```python
from build123d import *

# Parameters (mm, degrees)
EXTRUDE_1_DEPTH    = 100
SKETCH_2_W         = 6
SKETCH_2_H         = 1
EXTRUDE_2_DEPTH    = 100
HOLE_WIZARD_M3_1_D = 3.4


with BuildPart() as part:
    # 草图1 → 拉伸-薄壁1 (new body)
    with BuildSketch(Plane.XY):
        Polygon((2.35, 5), (0, 5), (0, 0), (8, 0), (8, 5), (5.65, 5), (5.65, 4), (7, 4), (7, 1), (1, 1), (1, 4), (2.35, 4), align=None)
    extrude(amount=EXTRUDE_1_DEPTH)

    # 草图2 → 拉伸-薄壁2 (add)
    with BuildSketch(Plane.XY.offset(100)):
        with Locations((-3, 0.5)):
            Rectangle(SKETCH_2_W, SKETCH_2_H)
    extrude(amount=-EXTRUDE_2_DEPTH)

    # 镜向1: part across plane


with BuildPart() as part_1:
    add(part.part)
    add(part.part.mirror(Plane(origin=(-6, 0, -6.08276253), x_dir=(0, 0, 1), z_dir=(1, 0, 0))))

    # M3 间隙孔1 (through all)
    with Locations(Plane(origin=(0, 1, 0), x_dir=(1, 0, 0), z_dir=(0, 1, 0))):
        with Locations((-6, -90), (-6, -10)):
            Hole(HOLE_WIZARD_M3_1_D / 2)


solid = part_1.part
```
Geometry check sheet. Reference: the model listing, model coordinates, mm. A direction names the side the tool comes from. Round coordinates to 2 decimals unless told otherwise and drop trailing zeros. Loops run counter-clockwise (first coordinate to the right, second up) from the corner with the lowest first, then second, coordinate; pieces in that order, holes last. Notation, with made-up numbers: M 85,-29 L 107,-29 A16 ccw 107,-22 Z; hole C 37.5,61.5 d9. An arc over 180 degrees is marked long. Return JSON: item names as keys, results as strings. Group by question number.
(1) Section check D-D, the plane x = 3.5. Enter the section's corners in (y, z), and give its area (3 significant figures).
(2) Section check C-C, the plane z = 79. Enter the section's corners in (x, y), and give its area (3 significant figures).
(3) Scan lines: line 1 along X through (y, z) = (3.65, 59); line 2 along Z through (x, y) = (-6, 0.75); line 3 along X through (y, z) = (4.25, 11.5). Record each from-to range of solid material in increasing order. Write a range as [from, to].
(4) Set-up check for faces 1 (the face through (0, 3, 49)), 2 (the face through (-19, 3, 49)), 3 (the face through (-5.8, 0.3, 0)): record each of +Z, -Z, +X, -X, +Y, -Y from which the full face is reachable in a straight line by a thin tool's end or side.
(5) Mould release check, pull along Y, two halves, no side actions. Record for faces 4 (the face through (-16, 1, 49)), 5 (the face through (1, 5, 49)), 6 (the face through (-5.63, 0.49, 91.66)): pulls with the +Y half, pulls with the -Y half, needs draft (parallel to the pull), parting line crosses it, or undercut.
(6) Section check A-A, the plane x = -6. Enter the section's corners in (y, z).
(7) Go/stop test with a flat-tipped pin: pin 1 (1.8 mm diameter, centred on x = -15.5, z = 55.5, fed in from +Y). Record where the tip stops, or that it passes through.
(8) Section check B-B, the plane z = 10. Enter the section's corners in (x, y), and give its area (3 significant figures).
Data:
{
 "1": {"outline": "M 0,0 L 1,0 L 1,100 L 0,100 Z", "area": "100 mm²"},
 "2": {"outline": "M -20,0 L 8,0 L 8,5 L 5.65,5 L 5.65,4 L 7,4 L 7,1 L 1,1 L 1,4 L 2.35,4 L 2.35,5 L 0,5 L 0,1 L -12,1 L -12,5 L -14.35,5 L -14.35,4 L -13,4 L -13,1 L -19,1 L -19,4 L -17.65,4 L -17.65,5 L -20,5 Z", "area": "49.4 mm²"},
 "3": {"line 1": "[-20, -19], [-13, -12], [0, 1], [7, 8]", "line 2": "[0, 8.3], [11.7, 88.3], [91.7, 100]", "line 3": "[-20, -17.65], [-14.35, -12], [0, 2.35], [5.65, 8]"},
 "4": {"face 1": "+Z, -Z, +Y", "face 2": "+Z, -Z", "face 3": "-Z, +X, -X, +Y, -Y"},
 "5": {"face 4": "undercut", "face 5": "pulls with the +Y half", "face 6": "needs draft"},
 "6": {"outline": "M 0,0 L 1,0 L 1,8.3 L 0,8.3 Z; M 0,11.7 L 1,11.7 L 1,88.3 L 0,88.3 Z; M 0,91.7 L 1,91.7 L 1,100 L 0,100 Z"},
 "7": {"pin 1": "y = 1"},
 "8": {"outline": "M -20,0 L -7.7,0 L -7.7,1 L -12,1 L -12,5 L -14.35,5 L -14.35,4 L -13,4 L -13,1 L -19,1 L -19,4 L -17.65,4 L -17.65,5 L -20,5 Z; M -4.3,0 L 8,0 L 8,5 L 5.65,5 L 5.65,4 L 7,4 L 7,1 L 1,1 L 1,4 L 2.35,4 L 2.35,5 L 0,5 L 0,1 L -4.3,1 Z", "area": "46.0 mm²"}
}
